from build123d import *


with BuildPart() as part:
    # Sketch1 → Revolve1 (revolve)
    with BuildSketch(Plane.XY, mode=Mode.PRIVATE) as revolve1_sk:
        Polygon((0, 0), (-3, 0), (-3, -9.5), (-2.675, -12), (-2.675, -20), (-3, -22.5), (-3, -30), (0, -30), align=None)
    revolve(revolve1_sk.sketch.rotate(Axis((0, -30, 0), (0, 1, 0)), 270), axis=Axis((0, -30, 0), (0, 1, 0)))


solid = part.part
Read the model definition and answer for the solid it produces. Units are mm, in the model's axes. A direction names the side the tool comes from. Give positions to 0.01 mm unless a question says otherwise; leave off trailing zeros. Write each loop counter-clockwise with the first axis right and the second up, starting at its lowest first coordinate (ties: lowest second). Pieces come first, ordered by that corner, then holes. Notation, with made-up numbers: (-14, -24.75) -> (10, -24.75) arc R16 cw to (10, -16.75) -> close; hole circle Ø10 at (19, 87). An arc over 180 degrees is marked (long way). Answer as a JSON object with one key per item and string values. Group by question number.
1) The mould has two halves that part along Y. Classify faces 1 (the cylindrical face through (-0.9, -4.82, -2.86)), 2 (the flat face through (0, -30, 0)), 3 (the conical face through (-0.842, -20.99, -2.674)): +Y half, -Y half, draft (parallel to the pull), parting line (faces both ways), or undercut.
2) Consider L1, parallel to X at y = -1.25, z = 1.3; L2, parallel to Z at x = -2.15, y = -24; L3, parallel to X at y = -5, z = -2.5. Determine where each line is inside the solid, lowest interval first. Write a range as from..to.
3) Find section A-A (z = 0). Write down the section's boundary in (x, y) (3 decimals), and give its area (3 significant figures).
4) Find section B-B (x = 0). Write down the section's boundary in (y, z) (3 decimals), and give its area (3 significant figures).
5) Find section C-C (y = -20.5). Write down the section's boundary in (x, z).
6) Find section D-D (y = -17). Write down the section's boundary in (x, z) (3 decimals).
7) Each of these flat-tipped pins is pushed along its axis until it touches: P1, Ø1, axis at x = 1, y = -17.5, coming from the +Z side; P2, Ø2, axis at y = -19, z = 1.5, coming from the +X side. Where does it stop, or does it pass through?
8) A tool of negligible diameter and unlimited length cuts with its end or side. For faces 4 (the cylindrical face through (2.61, -16.06, 0.58)), 5 (the cylindrical face through (-0.9, -26.3, -2.86)), from which of +Z, -Z, +X, -X, +Y, -Y can it reach the whole face along a straight path? Write none if from no direction.
Values follow:
{
 "1": {"face 1": "draft", "face 2": "-Y half", "face 3": "undercut"},
 "2": {"L1": "x = -2.7..2.7", "L2": "z = -2.09..2.09", "L3": "x = -1.66..1.66"},
 "3": {"outline": "(-3, -30) -> (3, -30) -> (3, -22.5) -> (2.675, -20) -> (2.675, -12) -> (3, -9.5) -> (3, 0) -> (-3, 0) -> (-3, -9.5) -> (-2.675, -12) -> (-2.675, -20) -> (-3, -22.5) -> close", "area": "173 mm2"},
 "4": {"outline": "(-30, -3) -> (-22.5, -3) -> (-20, -2.675) -> (-12, -2.675) -> (-9.5, -3) -> (0, -3) -> (0, 3) -> (-9.5, 3) -> (-12, 2.675) -> (-20, 2.675) -> (-22.5, 3) -> (-30, 3) -> close", "area": "173 mm2"},
 "5": {"outline": "circle Ø5.48 at (0, 0)"},
 "6": {"outline": "circle Ø5.35 at (0, 0)"},
 "7": {"P1": "stops at z = 2.63", "P2": "stops at x = 2.63"},
 "8": {"face 4": "none", "face 5": "+Y, -Y"}
}
